The model under review builds one solid part; all positions refer to its coordinate system, in mm. A direction names the side the tool comes from. Give positions to 0.01 mm unless a question says otherwise; leave off trailing zeros. Loops run counter-clockwise (first coordinate to the right, second up) from the corner with the lowest first, then second, coordinate; pieces in that order, holes last. Notation, with made-up numbers: M 46,46 L 66,46 A36 ccw 66,84 Z; hole C -7,-6.75 d11. An arc over 180 degrees is marked long. Return JSON: item names as keys, results as strings. Group by question number.
```python
from build123d import *

# Parameters (mm, degrees)
SKETCH_1_R             = 6
EXTRUDE_1_DEPTH        = 90
PATTERN_LINEAR_1_COUNT = 2
PATTERN_LINEAR_1_PITCH = 51.1
HOLE_WIZARD_M6_1_D     = 5
HOLE_WIZARD_M6_1_DEPTH = 11
HOLE_WIZARD_M6_1_TIP   = 1.502151548


with BuildPart() as part:
    # 草图1 → 凸台-拉伸1 (new body)
    with BuildSketch(Plane.XY):
        with Locations(Location((0, 0, 0), (0, 0, 180))):
            Circle(SKETCH_1_R)
    extrude(amount=EXTRUDE_1_DEPTH)

    # Groove Sketch → Retaining Ring Groove (revolve, cut)
    with BuildSketch(Plane(origin=(4.683915956, 3.689622128, 8.399116992), x_dir=(-0.5195228612321346, -0.40923941910457057, 0.7500793921366791), z_dir=(0.6187960743401806, -0.785551664998033, 0)), mode=Mode.PRIVATE) as retaining_ring_groove_sk:
        with BuildLine():
            Line((67.563324222, -43.809060949), (67.655912914, -43.704049834))
            Line((67.655912914, -43.704049834), (66.830825582, -42.97656726))
            Line((66.830825582, -42.97656726), (66.738236891, -43.081578375))
            ThreePointArc((66.738236891, -43.081578375), (66.710962353, -43.161228331), (66.747997367, -43.236835366))
            Line((66.747997367, -43.236835366), (67.408067232, -43.818821425))
            ThreePointArc((67.408067232, -43.818821425), (67.487717188, -43.846095963), (67.563324222, -43.809060949))
        make_face()
    retaining_ring_groove = revolve(retaining_ring_groove_sk.sketch.rotate(Axis((0, 0, 41.519998945), (0, 0, -1)), 128.228270648), axis=Axis((0, 0, 41.519998945), (0, 0, -1)), mode=Mode.SUBTRACT)

    # 阵列(线性)1: Retaining Ring Groove ×2
    with Locations(*[(0, 0, -i * PATTERN_LINEAR_1_PITCH) for i in range(1, PATTERN_LINEAR_1_COUNT)]):
        add(retaining_ring_groove, mode=Mode.SUBTRACT)

    # M6 螺纹孔1
    with Locations(Plane(origin=(0, 0, 0), x_dir=(-1, 0, 0), z_dir=(0, 0, -1))):
        with Locations((0, 0)):
            Hole(HOLE_WIZARD_M6_1_D / 2, depth=HOLE_WIZARD_M6_1_DEPTH)
            with Locations((0, 0, -(HOLE_WIZARD_M6_1_DEPTH + HOLE_WIZARD_M6_1_TIP / 2))):  # 118° drill point
                Cone(0, HOLE_WIZARD_M6_1_D / 2, HOLE_WIZARD_M6_1_TIP, mode=Mode.SUBTRACT)


solid = part.part
```
(1) Mouldability with a two-part tool opening along Z and no side actions: class faces 1 (the cylindrical face through (-5.723, -1.802, 89.011)), 2 (the cylindrical face through (1.727, 5.484, 87.506)), 3 (the conical face through (0.094, -0.424, 12.241)), 4 (the cylindrical face through (1.727, 5.484, 36.406)) as released by +Z, released by -Z, zero draft, split by the parting line, or undercut.
(2) For pin 1 (3.5 mm diameter, centred on x = -0.5, y = 0, fed in from -Z); pin 2 (1 mm diameter, centred on y = 3, z = 73.5, fed in from +X); pin 3 (1.5 mm diameter, centred on x = -2, z = 53, fed in from -Y), all flat-tipped, find the tip position at first contact; note any pin that passes through.
(3) Add section A-A (z = 48). Write out the cut boundary in (x, y).
(4) For faces 5 (the flat face through (0, 0, 90)), 6 (the cylindrical face through (-0.54, -2.44, 5.58)), list the 3-axis set-ups (+Z, -Z, +X, -X, +Y, -Y) from which the entire face can be reached by the end or side of a thin tool; tool diameter is ignored.
(5) For probe 1 along Y at (x, z) = (0, 5); probe 2 along Y at (x, z) = (-0.25, 57); probe 3 along Z at (x, y) = (0, 2.25), list the stretches that pass through material, from the lowest coordinate up.
Verdict:
{
 "1": {"face 1": "zero draft", "face 2": "undercut", "face 3": "released by -Z", "face 4": "undercut"},
 "2": {"pin 1": "stops at z = 11.15", "pin 2": "stops at x = 5.45", "pin 3": "stops at y = -5.87"},
 "3": {"outline": "C 0,0 d12"},
 "4": {"face 5": "+Z, +X, -X, +Y, -Y", "face 6": "-Z"},
 "5": {"probe 1": "y = -6 to -2.5, 2.5 to 6", "probe 2": "y = -5.99 to 5.99", "probe 3": "z = 11.15 to 90"}
}
